Part model, mm, in its own coordinate system. Face numbers are marked on the shaded views. A direction names the side the tool comes from. Coordinates: 2 decimals unless noted, no trailing zeros. Loops run counter-clockwise (first coordinate to the right, second up) from the corner with the lowest first, then second, coordinate; pieces in that order, holes last.
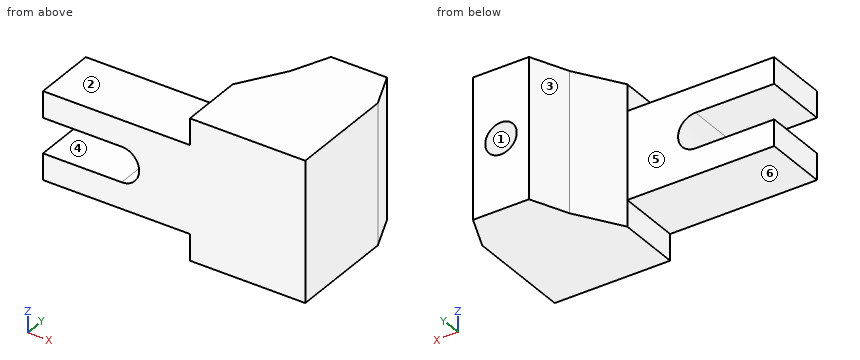
```python
from build123d import *

# Parameters (mm, degrees)
MAIN_BLOCK_DEPTH      = 80
BLOCK_EXTENSION_DEPTH = 80
HOLE_18_SKETCH_R      = 9
THROUGH_HOLE_18_DEPTH = 80
SLOTTED_ARM_DEPTH     = 36


with BuildPart() as part:
    # Main Block Profile → Main Block (new body)
    with BuildSketch(Plane.XY):
        Polygon((0, 0), (66, 0), (66, 61), (16, 61), (0, 36), align=None)
    extrude(amount=MAIN_BLOCK_DEPTH)

    # Block Extension Profile → Block Extension (add)
    with BuildSketch(Plane.XY.offset(80)):
        Polygon((41, 82), (57, 82), (66, 61), (16, 61), (25, 82), align=None)
    extrude(amount=-BLOCK_EXTENSION_DEPTH)

    # Hole Ø18 Sketch → Through Hole Ø18 (cut)
    with BuildSketch(Plane(origin=(0, 82, 0), x_dir=(1, 0, 0), z_dir=(0, 1, 0))):
        with Locations(Location((41, -40, 0), (0, 0, 270))):
            Circle(HOLE_18_SKETCH_R)
    extrude(amount=-THROUGH_HOLE_18_DEPTH, mode=Mode.SUBTRACT)

    # Slotted Arm Profile → Slotted Arm (add)
    with BuildSketch(Plane.XZ):
        with BuildLine():
            Line((0, 65), (0, 15))
            Line((0, 15), (-84, 15))
            Line((-84, 15), (-84, 30))
            Line((-84, 30), (-39, 30))
            ThreePointArc((-39, 30), (-29, 40), (-39, 50))
            Line((-39, 50), (-84, 50))
            Line((-84, 50), (-84, 65))
            Line((-84, 65), (0, 65))
        make_face()
    extrude(amount=-SLOTTED_ARM_DEPTH)


solid = part.part
```
Q1. Saw through at D-D (x = 41). List the corners of the cut face in (y, z), plus the area to 3 significant figures.
Q2. Saw through at C-C (z = 6). List the corners of the cut face in (x, y).
Q3. Saw through at A-A (x = -46.5). List the corners of the cut face in (y, z).
Q4. Mould opens along Z. For the marked faces 1, 2 and 3 say: released by +Z, released by -Z, zero draft, split by the parting line, or undercut.
Q5. Drop flat-ended pins along their axis: P1, Ø23.5, axis at x = 41, z = 40, coming from the +Y side; P2, Ø3, axis at y = 53.5, z = 53.5, coming from the -X side; P3, Ø8, axis at y = 49, z = 37.5, coming from the -X side; P4, Ø18, axis at x = -36.5, y = 20.5, coming from the -Z side. Give the stop position or say it passes through.
Q6. Saw through at B-B (y = 17.5). List the corners of the cut face in (x, z).
Q7. Tool access for the marked faces 4, 5 and 6: list every direction of +Z, -Z, +X, -X, +Y, -Y with a clear straight run to the whole face (end or side of a thin tool).
Q8. Probe line 1 (X direction, y = 18.5, z = 40); line 2 (Y direction, x = -33, z = 64.5); line 3 (Z direction, x = -49.5, y = 19). List the from-to ranges inside material, lowest first.
Checked values:
1. outline: (0, 0) - (82, 0) - (82, 31) - (2, 31) - (2, 49) - (82, 49) - (82, 80) - (0, 80) - close
1. area: 5,120 mm2
2. outline: (0, 0) - (66, 0) - (66, 61) - (57, 82) - (25, 82) - (16, 61) - (0, 36) - close
3. outline: (0, 15) - (36, 15) - (36, 30) - (0, 30) - close; (0, 50) - (36, 50) - (36, 65) - (0, 65) - close
4. face 1: undercut
4. face 2: released by +Z
4. face 3: zero draft
5. P1: stops at y = 82
5. P2: stops at x = 10.24
5. P3: stops at x = 5.76
5. P4: stops at z = 15
6. outline: (-84, 15) - (0, 15) - (0, 0) - (66, 0) - (66, 80) - (0, 80) - (0, 65) - (-84, 65) - (-84, 50) - (-39, 50) arc R10 cw to (-39, 30) - (-84, 30) - close; hole circle Ø18 at (41, 40)
7. face 4: -X, +Y, -Y
7. face 5: +Z, -Z, -X, +Y
7. face 6: -Z, -X, +Y, -Y
8. line 1: x = -29 to 32, 50 to 66
8. line 2: y = 0 to 36
8. line 3: z = 15 to 30, 50 to 65
